```python
from build123d import *

# Parameters (mm, degrees)
SKETCH1_R           = 8
BOSS_EXTRUDE1_DEPTH = 231.7
SKETCH2_R           = 6
BOSS_EXTRUDE2_DEPTH = 30
BOSS_EXTRUDE3_START = 70
SKETCH4_R           = 6
BOSS_EXTRUDE3_DEPTH = 70


with BuildPart() as part:
    # Sketch1 → Boss-Extrude1 (new, symmetric)
    with BuildSketch(Plane.XY):
        with Locations(Location((0, 0, 0), (0, 0, 180))):
            Circle(SKETCH1_R)
    extrude(amount=BOSS_EXTRUDE1_DEPTH, both=True)

    # Sketch2 → Boss-Extrude2 (add)
    with BuildSketch(Plane.XY.offset(231.7)):
        Circle(SKETCH2_R)
    extrude(amount=BOSS_EXTRUDE2_DEPTH)

    # Sketch4 → Boss-Extrude3 (add)
    with BuildSketch(Plane(origin=(0, 0, -231.7), x_dir=(-1, 0, 0), z_dir=(0, 0, -1)).offset(BOSS_EXTRUDE3_START)):
        with Locations(Location((0, 0, 0), (0, 0, 180))):
            Circle(SKETCH4_R)
    extrude(amount=-BOSS_EXTRUDE3_DEPTH)


solid = part.part
```
Source: CAD feature listing. Evaluate the final solid. Frame: model axes, mm. A direction names the side the tool comes from. Give positions to 0.01 mm unless a question says otherwise; leave off trailing zeros. Order: outer loops, then holes, each group sorted by start corner. A loop starts at its lowest first (then second) coordinate and runs counter-clockwise, first axis right, second up.
(1) Access query for faces 1 (the face through (1.73, 7.81, 3.24)), 2 (the face through (5.723, -1.802, -267.19)), 3 (the face through (2, -6, 231.7)). Directions: +Z, -Z, +X, -X, +Y, -Y. A direction counts if a zero-diameter tool reaches every point of the face in a straight line with its end or side. Return the directions, or none.
(2) Section query C-C (z = 61.5). Return the cut outline in (x, y).
(3) Section query B-B (x = 2.25). Return the cut outline in (y, z), plus the area to 3 significant figures.
(4) Section query A-A (y = 0). Return the cut outline in (x, z), plus the area to 3 significant figures.
(5) Contact query for flat-ended pins moving along their axis: P1, Ø1.5, axis at x = -1.5, z = -235, coming from the +Y side; P2, Ø8, axis at y = -4.5, z = 128, coming from the +X side; P3, Ø1, axis at y = -1, z = -117.5, coming from the -X side. Output: stop coordinate, or through.
(6) Material intervals for line 1 along Z through (x, y) = (-4.75, -6); line 2 along Y through (x, z) = (0.5, -27.5); line 3 along Y through (x, z) = (3.75, -82), sorted ascending.
Outcome:
1. face 1: +Z, -Z
1. face 2: -Z
1. face 3: +Z
2. outline: circle Ø16 at (0, 0)
3. outline: (-7.68, -231.7) - (-5.56, -231.7) - (-5.56, -301.7) - (5.56, -301.7) - (5.56, -231.7) - (7.68, -231.7) - (7.68, 231.7) - (5.56, 231.7) - (5.56, 261.7) - (-5.56, 261.7) - (-5.56, 231.7) - (-7.68, 231.7) - close
3. area: 8,230 mm2
4. outline: (-8, -231.7) - (-6, -231.7) - (-6, -301.7) - (6, -301.7) - (6, -231.7) - (8, -231.7) - (8, 231.7) - (6, 231.7) - (6, 261.7) - (-6, 261.7) - (-6, 231.7) - (-8, 231.7) - close
4. area: 8,610 mm2
5. P1: stops at y = 5.95
5. P2: stops at x = 7.98
5. P3: stops at x = -7.98
6. line 1: z = -231.7 to 231.7
6. line 2: y = -7.98 to 7.98
6. line 3: y = -7.07 to 7.07
